The drawing under review shows one solid part. Ordinate dimensions are in mm from its lowest x, y, z. Coordinates: 2 decimals unless noted, no trailing zeros. Order: outer loops, then holes, each group sorted by start corner. A loop starts at its lowest first (then second) coordinate and runs counter-clockwise, first axis right, second up. Notation, with made-up numbers: (70.5, 43) - (99.5, 43) arc R21 cw to (99.5, 59) - close; hole circle Ø9 at (65.5, 42.25). An arc over 180 degrees is marked (long way). Answer in a Markdown table with one row per item.
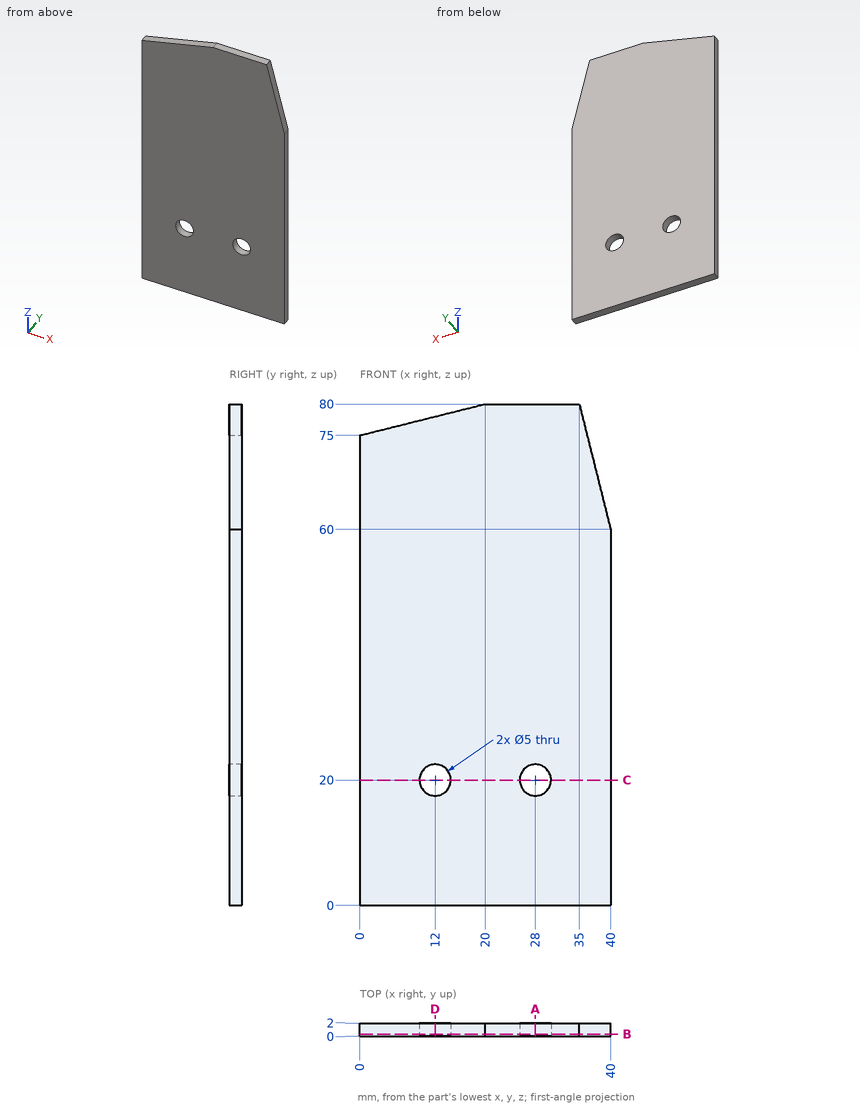
Item 1: We need section D-D, the plane x = 12. Write out the cut boundary in (y, z), then the cut area to 3 significant figures.
Check values:
| item | result |
|---|---|
| outline | (0, 0) - (2, 0) - (2, 17.5) - (0, 17.5) - close; (0, 22.5) - (2, 22.5) - (2, 78) - (0, 78) - close |
| area | 146 mm^2 |
Item 2: We need section C-C, the plane z = 20. Write out the cut boundary in (x, y).
Check values:
| item | result |
|---|---|
| outline | (0, 0) - (9.5, 0) - (9.5, 2) - (0, 2) - close; (14.5, 0) - (25.5, 0) - (25.5, 2) - (14.5, 2) - close; (30.5, 0) - (40, 0) - (40, 2) - (30.5, 2) - close |
Item 3: Clearance check with a flat-ended pin moving along its axis: pin 1 Ø3 at (x, z) = (12, 20) entering from +Y. State where the tip first meets the part, or that it passes through.
Check values:
| item | result |
|---|---|
| pin 1 | through |
Item 4: We need section B-B, the plane y = 0.3. Write out the cut boundary in (x, z), then the cut area to 3 significant figures.
Check values:
| item | result |
|---|---|
| outline | (0, 0) - (40, 0) - (40, 60) - (35, 80) - (20, 80) - (0, 75) - close; hole circle Ø5 at (12, 20); hole circle Ø5 at (28, 20) |
| area | 3,060 mm^2 |
Item 5: We need section A-A, the plane x = 28. Write out the cut boundary in (y, z), then the cut area to 3 significant figures.
Check values:
| item | result |
|---|---|
| outline | (0, 0) - (2, 0) - (2, 17.5) - (0, 17.5) - close; (0, 22.5) - (2, 22.5) - (2, 80) - (0, 80) - close |
| area | 150 mm^2 |
Item 6: To check wall thickness, follow line 1 (X direction, y = 1, z = 20); line 2 (X direction, y = 1.75, z = 19.5); line 3 (Z direction, x = 10, y = 0.1). State the ranges of each line that lie inside material, in increasing order. Write a range as from..to.
Check values:
| item | result |
|---|---|
| line 1 | 0..9.5, 14.5..25.5, 30.5..40 |
| line 2 | 0..9.55, 14.45..25.55, 30.45..40 |
| line 3 | 0..18.5, 21.5..77.5 |
